from build123d import *

# Parameters (mm, degrees)
SKETCH1_W                                 = 15
SKETCH1_H                                 = 40
BOSS_EXTRUDE1_DEPTH                       = 25
FILLET1_R                                 = 5
HOLE_WIZARD_SOCKET_HEAD_CAP_SCREW_2_COUNT = 2
HOLE_WIZARD_SOCKET_HEAD_CAP_SCREW_2_PITCH = 20


with BuildPart() as part:
    # Sketch1 → Boss-Extrude1 (new body)
    with BuildSketch(Plane(origin=(0, 0, 0), x_dir=(1, 0, 0), z_dir=(0, 1, 0))):
        Rectangle(SKETCH1_W, SKETCH1_H)
    extrude(amount=BOSS_EXTRUDE1_DEPTH)

    # Fillet1
    fillet1_edges = [part.edges().sort_by_distance(p)[0] for p in [
        (7.5, 12.5, 20),
        (7.5, 12.5, -20),
    ]]
    fillet(fillet1_edges, radius=FILLET1_R)

    # Sketch3 → Hole wizard: socket head cap screw, type 1 (revolve, cut)
    with BuildSketch(Plane(origin=(0, 25, -10), x_dir=(0, 0, 1), z_dir=(1, 0, 0))):
        Polygon((0, 0), (0, 25), (2.25, 25), (2.25, 4.6), (4, 4.6), (4, 0.025), (4.025, 0), align=None)
    hole_wizard_socket_head_cap_screw_type = revolve(axis=Axis((0, 31.35, -10), (0, -1, 0)), mode=Mode.SUBTRACT)

    # Hole wizard_ socket head cap screw_  2: Hole wizard: socket head cap screw, type 1 ×2
    with Locations(*[(0, 0, i * HOLE_WIZARD_SOCKET_HEAD_CAP_SCREW_2_PITCH) for i in range(1, HOLE_WIZARD_SOCKET_HEAD_CAP_SCREW_2_COUNT)]):
        add(hole_wizard_socket_head_cap_screw_type, mode=Mode.SUBTRACT)


solid = part.part
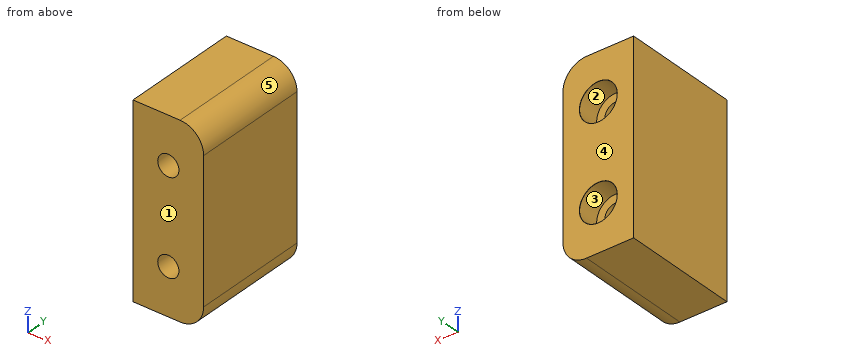
Check sheet for the modelled part. Datum: model origin and axes. Units: mm. Face numbers are marked on the shaded views. A direction names the side the tool comes from. Round coordinates to 2 decimals unless told otherwise and drop trailing zeros. Loops run counter-clockwise (first coordinate to the right, second up) from the corner with the lowest first, then second, coordinate; pieces in that order, holes last. Notation, with made-up numbers: (-24.75, 58.25) - (30.25, 58.25) arc R21 ccw to (30.25, 80.25) - close; hole circle Ø8 at (47, 54.5). An arc over 180 degrees is marked (long way). Answer as CSV lines item,"result". Start each with the question number.
Item 1: Section check B-B (x = 0). Record the boundary of the cut face in (y, z) (3 decimals), and give its area (3 significant figures).
Item 2: Set-up check for the marked faces 1 and 2: record each of +Z, -Z, +X, -X, +Y, -Y from which the full face is reachable in a straight line by a thin tool's end or side.
Item 3: Section check D-D (x = 5.5). Record the boundary of the cut face in (y, z).
Item 4: Depth check by flat-ended pin: P1, Ø1.5, axis at x = 4, y = 20.5, coming from the +Z side; P2, Ø6.5, axis at x = -0.5, z = 9.5, coming from the +Y side. Enter the tip coordinate at first touch or a pass-through.
Item 5: Section check A-A (z = 10). Record the boundary of the cut face in (x, y) (3 decimals), and give its area (3 significant figures).
Item 6: Scan lines: line 1 (Z direction, x = 0, y = 21.3); line 2 (Z direction, x = 0, y = 11.5); line 3 (X direction, y = 21.9, z = -10). Record each from-to range of solid material in increasing order. Write a range as [from, to].
Item 7: Section check C-C (y = 10.25). Record the boundary of the cut face in (x, z).
Item 8: Release check for a two-part mould opening along X. For the marked faces 3, 4 and 5 record: +X half, -X half, draft (parallel to the pull), parting line (faces both ways), or undercut.
Report:
1,outline,"(0, -20) - (25, -20) - (25, -14.025) - (24.975, -14) - (20.4, -14) - (20.4, -12.25) - (0, -12.25) - close; (0, -7.75) - (20.4, -7.75) - (20.4, -6) - (24.975, -6) - (25, -5.975) - (25, 5.975) - (24.975, 6) - (20.4, 6) - (20.4, 7.75) - (0, 7.75) - close; (0, 12.25) - (20.4, 12.25) - (20.4, 14) - (24.975, 14) - (25, 14.025) - (25, 20) - (0, 20) - close"
1,area,"743 mm2"
2,face 1,"+Z, -Z, +X, -X, -Y"
2,face 2,"+Y"
3,outline,"(0, -19) - (25, -19) - (25, 19) - (0, 19) - close"
4,P1,"stops at z = 19.94"
4,P2,"stops at y = 20.4"
5,outline,"(-7.5, 0) - (-2.25, 0) - (-2.25, 20.4) - (-4, 20.4) - (-4, 24.975) - (-4.025, 25) - (-7.5, 25) - close; (2.25, 0) - (7.5, 0) - (7.5, 25) - (4.025, 25) - (4, 24.975) - (4, 20.4) - (2.25, 20.4) - close"
5,area,"246 mm2"
6,line 1,"z = [-20, -14], [-6, 6], [14, 20]"
6,line 2,"z = [-20, -12.25], [-7.75, 7.75], [12.25, 20]"
6,line 3,"x = [-7.5, -4], [4, 7.5]"
7,outline,"(-7.5, -20) - (2.5, -20) arc R5 ccw to (7.5, -15) - (7.5, 15) arc R5 ccw to (2.5, 20) - (-7.5, 20) - close; hole circle Ø4.5 at (0, -10); hole circle Ø4.5 at (0, 10)"
8,face 3,"undercut"
8,face 4,"draft"
8,face 5,"+X half"
